Build history of the part. All positions in model axes, mm. A direction names the side the tool comes from. Round coordinates to 2 decimals unless told otherwise and drop trailing zeros. Loops run counter-clockwise (first coordinate to the right, second up) from the corner with the lowest first, then second, coordinate; pieces in that order, holes last. Notation, with made-up numbers: M -6.5,41 L 11.5,41 A27 ccw 11.5,65 Z; hole C 31.5,9 d3. An arc over 180 degrees is marked long. One line per item, written item: value.
```python
from build123d import *

# Parameters (mm, degrees)
BRACKET_BODY_DEPTH      = 42
TOP_SLOT_CUT_DEPTH      = 10
THROUGH_SLOT_10MM_DEPTH = 42
SLOT_RELIEF_SKETCH_W    = 6
SLOT_RELIEF_SKETCH_H    = 10
SLOT_RELIEF_CUT_DEPTH   = 42
SIDE_BOSS_A_SKETCH_W    = 80
SIDE_BOSS_A_SKETCH_H    = 40
SIDE_BOSS_A_DEPTH       = 10
SIDE_BOSS_B_SKETCH_W    = 80
SIDE_BOSS_B_SKETCH_H    = 40
SIDE_BOSS_B_DEPTH       = 10
CORNER_ROUND_R24_R      = 24
ARCH_CUTOUT_DEPTH       = 42
NOTCH_SKETCH_W          = 8
NOTCH_SKETCH_H          = 22
NOTCH_CUT_DEPTH         = 42


with BuildPart() as part:
    # Bracket Profile Sketch → Bracket Body (new body)
    with BuildSketch(Plane.XY):
        with BuildLine():
            Line((-40, 0), (40, 0))
            Line((40, 0), (40, 10))
            Line((40, 10), (40, 16))
            ThreePointArc((40, 16), (32.970562748, 32.970562748), (16, 40))
            Line((16, 40), (6, 40))
            Line((6, 40), (-40, 40))
            Line((-40, 40), (-40, 0))
        make_face()
    extrude(amount=-BRACKET_BODY_DEPTH)

    # Top Slot Sketch → Top Slot Cut (cut)
    with BuildSketch(Plane(origin=(0, 40, 0), x_dir=(1, 0, 0), z_dir=(0, 1, 0))):
        with BuildLine():
            Line((-40, 23.147915888), (-17.706260918, 23.147915888))
            ThreePointArc((-17.706260918, 23.147915888), (-10, 29), (-2.293739082, 23.147915888))
            Line((-2.293739082, 23.147915888), (6, 23.147915888))
            Line((6, 23.147915888), (6, 17.147915888))
            Line((6, 17.147915888), (-2.988477484, 17.147915888))
            ThreePointArc((-2.988477484, 17.147915888), (-10, 13), (-17.011522516, 17.147915888))
            Line((-17.011522516, 17.147915888), (-40, 17.147915888))
            Line((-40, 17.147915888), (-40, 23.147915888))
        make_face()
    extrude(amount=-TOP_SLOT_CUT_DEPTH, mode=Mode.SUBTRACT)

    # Through Slot Sketch → Through Slot 10mm (cut)
    with BuildSketch(Plane.XY):
        with BuildLine():
            Line((6, 40), (40, 10))
            Line((40, 10), (40, 16))
            ThreePointArc((40, 16), (32.970562748, 32.970562748), (16, 40))
            Line((16, 40), (6, 40))
        make_face()
    extrude(amount=-THROUGH_SLOT_10MM_DEPTH, mode=Mode.SUBTRACT)

    # Slot Relief Sketch → Slot Relief Cut (cut)
    with BuildSketch(Plane.ZY.offset(-6)):
        with Locations((-20.147915888, 35)):
            Rectangle(SLOT_RELIEF_SKETCH_W, SLOT_RELIEF_SKETCH_H)
    extrude(amount=-SLOT_RELIEF_CUT_DEPTH, mode=Mode.SUBTRACT)

    # Side Boss A Sketch → Side Boss A (add)
    with BuildSketch(Plane.XY):
        with Locations((0, 20)):
            Rectangle(SIDE_BOSS_A_SKETCH_W, SIDE_BOSS_A_SKETCH_H)
    extrude(amount=-SIDE_BOSS_A_DEPTH)

    # Side Boss B Sketch → Side Boss B (add)
    with BuildSketch(Plane(origin=(0, 0, -42), x_dir=(-1, 0, 0), z_dir=(0, 0, -1))):
        with Locations((0, 20)):
            Rectangle(SIDE_BOSS_B_SKETCH_W, SIDE_BOSS_B_SKETCH_H)
    extrude(amount=-SIDE_BOSS_B_DEPTH)

    # Corner Round R24
    corner_round_r24_edges = [part.edges().sort_by_distance(p)[0] for p in [
        (40, 40, -37),
        (40, 40, -5),
    ]]
    fillet(corner_round_r24_edges, radius=CORNER_ROUND_R24_R)

    # Arch Cutout Sketch → Arch Cutout (cut)
    with BuildSketch(Plane.XY):
        with BuildLine():
            Line((-25, 0), (5, 0))
            ThreePointArc((5, 0), (-10, 15), (-25, 0))
        make_face()
    extrude(amount=-ARCH_CUTOUT_DEPTH, mode=Mode.SUBTRACT)

    # Notch Sketch → Notch Cut (cut)
    with BuildSketch(Plane(origin=(0, 40, 0), x_dir=(1, 0, 0), z_dir=(0, 1, 0))):
        with Locations((-36, 21)):
            Rectangle(NOTCH_SKETCH_W, NOTCH_SKETCH_H)
    extrude(amount=-NOTCH_CUT_DEPTH, mode=Mode.SUBTRACT)


solid = part.part
```
Item 1: Pull direction Z, two halves, no side cores. Call faces 1 (the face through (27, 30, -10)), 2 (the face through (40, 6, -21)), 3 (the face through (-10, 35, -29)), 4 (the face through (-1, 20, 0)): pulls with the +Z half, pulls with the -Z half, needs draft (parallel to the pull), parting line crosses it, or undercut.
Check values:
face 1: undercut
face 2: needs draft
face 3: undercut
face 4: pulls with the +Z half
Item 2: Slice it at B-B, the plane x = -10. Give the cut face in (y, z), and give its area (3 significant figures).
Check values:
outline: M 15,-42 L 40,-42 L 40,-29 L 30,-29 L 30,-13 L 40,-13 L 40,0 L 15,0 Z
area: 890 mm2
Item 3: Slice it at C-C, the plane z = -34.5. Give the cut face in (x, y), and give its area (3 significant figures).
Check values:
outline: M -40,0 L -25,0 A15 cw 5,0 L 40,0 L 40,16 A24 ccw 16,40 L -40,40 Z
area: 2,720 mm2
Item 4: Wall check: line 1 along Z through (x, y) = (-22.5, 33); line 2 along Z through (x, y) = (-35.5, 30); line 3 along X through (y, z) = (5, -4). Give the ranges that are in metal, low to high.
Check values:
line 1: z = -42 to -23.15, -17.15 to 0
line 2: z = -42 to -32, -10 to 0
line 3: x = -40 to -24.14, 4.14 to 40
Item 5: Drop flat-ended pins along their axis: P1, Ø6, axis at x = 28.5, z = -19.5, coming from the +Y side; P2, Ø1, axis at y = 18.5, z = -26, coming from the -X side; P3, Ø12, axis at x = 29, z = -8.5, coming from the +Y side. Give the stop position or say it passes through.
Check values:
P1: stops at y = 22.79
P2: stops at x = -32
P3: stops at y = 38.96
Item 6: Slice it at D-D, the plane y = 18.5. Give the cut face in (x, z).
Check values:
outline: M -40,-42 L 39.87,-42 L 39.87,-32 L 30.37,-32 L 30.37,-10 L 39.87,-10 L 39.87,0 L -40,0 L -40,-10 L -32,-10 L -32,-32 L -40,-32 Z
Item 7: Which spindle directions (+Z, -Z, +X, -X, +Y, -Y) get a long thin tool onto all of the face, cutting with end or side? Do faces 5 (the face through (-32, 20, -21)), 6 (the face through (27, 29, -32)), 7 (the face through (-24, 35, -17.148)), 8 (the face through (-1, 20, -42)). Say none if no direction does.
Check values:
face 5: -X, +Y, -Y
face 6: +X, +Y
face 7: +X, -X, +Y
face 8: -Z, +X, -X, +Y, -Y
Item 8: Slice it at A-A, the plane y = 31. Give the cut face in (x, z) (3 decimals).
Check values:
outline: M -40,-42 L 34.735,-42 L 34.735,-32 L 16.2,-32 L 16.2,-23.148 L -2.294,-23.148 A8 cw -17.706,-23.148 L -32,-23.148 L -32,-32 L -40,-32 Z; M -40,-10 L -32,-10 L -32,-17.148 L -17.012,-17.148 A8 cw -2.988,-17.148 L 16.2,-17.148 L 16.2,-10 L 34.735,-10 L 34.735,0 L -40,0 Z
